Here's how the part is built. I have some questions about the finished solid (model axes, mm). Face numbers are marked on the shaded views. A direction names the side the tool comes from. Give positions to 0.01 mm unless a question says otherwise; leave off trailing zeros. Write each loop counter-clockwise with the first axis right and the second up, starting at its lowest first coordinate (ties: lowest second). Pieces come first, ordered by that corner, then holes. Notation, with made-up numbers: M -18,5.5 L 10,5.5 A8 cw 10,15.5 Z; hole C -2.75,-7 d6. An arc over 180 degrees is marked long. Answer as CSV lines item,"result". Start each with the question number.
Q1. For pin 1 (13 mm diameter, centred on y = -12, z = 22.5, fed in from +X); pin 2 (6.5 mm diameter, centred on x = 20, z = 12, fed in from +Y), each with a flat end and sliding along its axis, tell me the tip position at first contact or that it passes through.
Q2. Suppose I cut it at B-B (z = 22.5). Write out the boundary of the cut face in (x, y).
Q3. Thinking about a two-plate mould opening in X: for the marked faces 3, 4, 5 and 6, which applies, +X half, -X half, draft (parallel to the pull), parting line (faces both ways), or undercut?
Q4. Suppose I cut it at A-A (y = -21). Write out the boundary of the cut face in (x, z).
Q5. On a 3-axis mill with a long thin cutter (end or side, diameter ignored), from which of +Z, -Z, +X, -X, +Y, -Y can I reach the whole of each face in a straight line? I mean the marked faces 1 and 2. Say none if no direction works.
Q6. Suppose I cut it at C-C (y = -12). Write out the boundary of the cut face in (x, z).
Q7. Suppose I cut it at D-D (z = 12.5). Write out the boundary of the cut face in (x, y).
Q8. If I drill on line 1 along X through (y, z) = (-29, 26); line 2 along Y through (x, z) = (30.95, 22.5); line 3 along Y through (x, z) = (25.5, 9.5), over which ranges is the centre line in solid material (lowest first)?
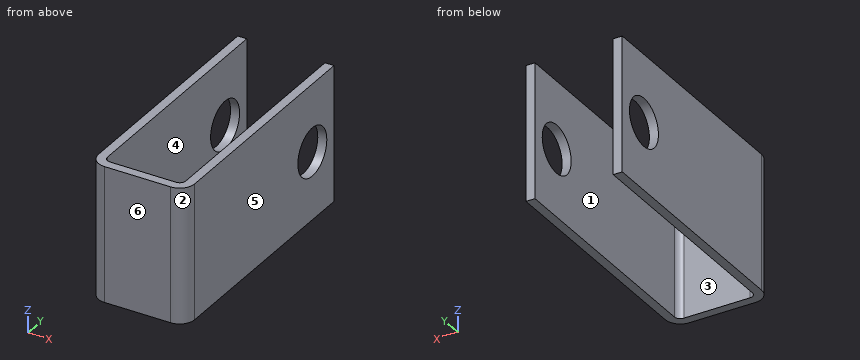
```python
from build123d import *

# Parameters (mm, degrees)
BOSS_EXTRUDE1_DEPTH = 45
SKETCH2_R           = 8
CUT_EXTRUDE1_DEPTH  = 99.858484714


with BuildPart() as part:
    # Sketch1 → Boss-Extrude1 (new body)
    with BuildSketch(Plane.XY):
        with BuildLine():
            Line((0, 0), (0, -77))
            ThreePointArc((0, -77), (1.464466094, -80.535533906), (5, -82))
            Line((5, -82), (27, -82))
            ThreePointArc((27, -82), (30.535533906, -80.535533906), (32, -77))
            Line((32, -77), (32, 0))
            Line((32, 0), (29, 0))
            Line((29, 0), (29, -77))
            ThreePointArc((29, -77), (28.414213562, -78.414213562), (27, -79))
            Line((27, -79), (5, -79))
            ThreePointArc((5, -79), (3.585786438, -78.414213562), (3, -77))
            Line((3, -77), (3, 0))
            Line((3, 0), (0, 0))
        make_face()
    extrude(amount=BOSS_EXTRUDE1_DEPTH)

    # Sketch2 → Cut-Extrude1 (cut, through all)
    with BuildSketch(Plane(origin=(32, 0, 0), x_dir=(0, 0, -1), z_dir=(1, 0, 0))):
        with Locations((-22.5, -12)):
            Circle(SKETCH2_R)
    extrude(amount=-CUT_EXTRUDE1_DEPTH, mode=Mode.SUBTRACT)


solid = part.part
```
Resolved:
1,pin 1,"through"
1,pin 2,"y = -79"
2,outline,"M 0,-77 A5 ccw 5,-82 L 27,-82 A5 ccw 32,-77 L 32,-20 L 29,-20 L 29,-77 A2 cw 27,-79 L 5,-79 A2 cw 3,-77 L 3,-20 L 0,-20 Z; M 0,-4 L 3,-4 L 3,0 L 0,0 Z; M 29,-4 L 32,-4 L 32,0 L 29,0 Z"
3,face 3,"undercut"
3,face 4,"undercut"
3,face 5,"+X half"
3,face 6,"draft"
4,outline,"M 0,0 L 3,0 L 3,45 L 0,45 Z; M 29,0 L 32,0 L 32,45 L 29,45 Z"
5,face 1,"+Z, -Z, +Y"
5,face 2,"+Z, -Z, +X, -Y"
6,outline,"M 0,0 L 3,0 L 3,14.5 L 0,14.5 Z; M 0,30.5 L 3,30.5 L 3,45 L 0,45 Z; M 29,0 L 32,0 L 32,14.5 L 29,14.5 Z; M 29,30.5 L 32,30.5 L 32,45 L 29,45 Z"
7,outline,"M 0,-77 A5 ccw 5,-82 L 27,-82 A5 ccw 32,-77 L 32,0 L 29,0 L 29,-77 A2 cw 27,-79 L 5,-79 A2 cw 3,-77 L 3,0 L 0,0 Z"
8,line 1,"0 to 3, 29 to 32"
8,line 2,"-80.07 to -20, -4 to 0"
8,line 3,"-82 to -79"
